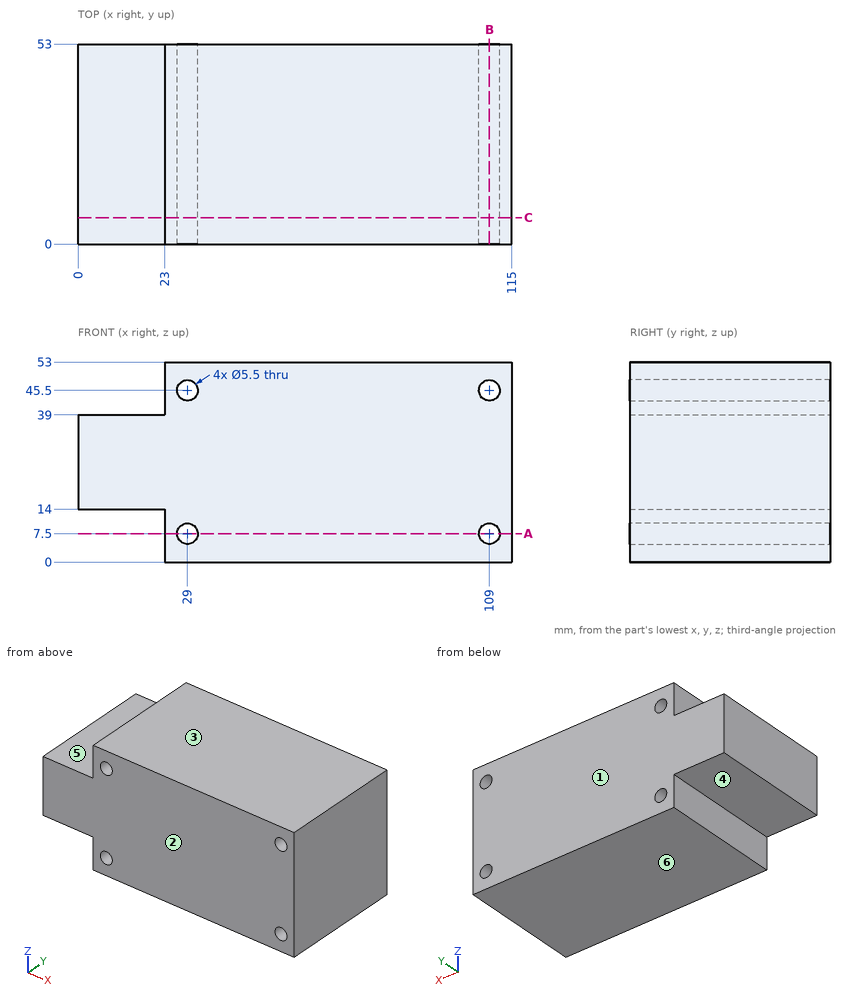
The figure shows three views and two pictorial views of one solid part (mm, origin at its lowest corner). Answer the questions. A direction names the side the tool comes from. Coordinates: 2 decimals unless noted, no trailing zeros. Loops run counter-clockwise (first coordinate to the right, second up) from the corner with the lowest first, then second, coordinate; pieces in that order, holes last. Notation, with made-up numbers: (-32, 32.25) - (-11, 32.25) arc R17 cw to (-11, 48.25) - close; hole circle Ø7 at (2.25, -24). An arc over 180 degrees is marked (long way). Use a Markdown table: item, result. Add a question column.
1) The part is cut by section A-A, the plane z = 7.5. Give the vertices of the cut face in (x, y), and give its area (3 significant figures).
2) The mould has two halves that part along Y. Classify the marked faces 1, 2 and 3: released by +Y, released by -Y, zero draft, split by the parting line, or undercut.
3) The part is cut by section B-B, the plane x = 109. Give the vertices of the cut face in (y, z).
4) The part is cut by section C-C, the plane y = 7. Give the vertices of the cut face in (x, z), and give its area (3 significant figures).
5) Given pin 1 (8 mm diameter, centred on x = 82.5, y = 30, fed in from -Z); pin 2 (8 mm diameter, centred on y = 44, z = 8, fed in from -X), each flat-ended and moving along its own axis, determine where each tip first touches the part or whether it passes through.
6) Find the intervals of material crossed by line 1 (Z direction, x = 109, y = 24); line 2 (X direction, y = 19.5, z = 45.5); line 3 (Z direction, x = 15, y = 32), in increasing order.
7) For the marked faces 4, 5 and 6, determine the directions among +Z, -Z, +X, -X, +Y, -Y from which every point of the face is accessible in a straight line to the end or side of a thin tool.
Here are the results:
| question | item | result |
|---|---|---|
| 1 | outline | (23, 0) - (26.25, 0) - (26.25, 53) - (23, 53) - close; (31.75, 0) - (106.25, 0) - (106.25, 53) - (31.75, 53) - close; (111.75, 0) - (115, 0) - (115, 53) - (111.75, 53) - close |
| 1 | area | 4,290 mm^2 |
| 2 | face 1 | released by +Y |
| 2 | face 2 | released by -Y |
| 2 | face 3 | zero draft |
| 3 | outline | (0, 0) - (53, 0) - (53, 4.75) - (0, 4.75) - close; (0, 10.25) - (53, 10.25) - (53, 42.75) - (0, 42.75) - close; (0, 48.25) - (53, 48.25) - (53, 53) - (0, 53) - close |
| 4 | outline | (0, 14) - (23, 14) - (23, 0) - (115, 0) - (115, 53) - (23, 53) - (23, 39) - (0, 39) - close; hole circle Ø5.5 at (29, 7.5); hole circle Ø5.5 at (29, 45.5); hole circle Ø5.5 at (109, 7.5); hole circle Ø5.5 at (109, 45.5) |
| 4 | area | 5,360 mm^2 |
| 5 | pin 1 | stops at z = 0 |
| 5 | pin 2 | stops at x = 23 |
| 6 | line 1 | z = 0 to 4.75, 10.25 to 42.75, 48.25 to 53 |
| 6 | line 2 | x = 23 to 26.25, 31.75 to 106.25, 111.75 to 115 |
| 6 | line 3 | z = 14 to 39 |
| 7 | face 4 | -Z, -X, +Y, -Y |
| 7 | face 5 | +Z, -X, +Y, -Y |
| 7 | face 6 | -Z, +X, -X, +Y, -Y |
